Work out the finished part from the listing and answer in its coordinate system (mm). A direction names the side the tool comes from. Coordinates: 2 decimals unless noted, no trailing zeros. Order: outer loops, then holes, each group sorted by start corner. A loop starts at its lowest first (then second) coordinate and runs counter-clockwise, first axis right, second up.
```python
from build123d import *

# Parameters (mm, degrees)
SKETCH1_W           = 180
SKETCH1_H           = 50
BOSS_EXTRUDE1_DEPTH = 10
SKETCH2_W           = 10
SKETCH2_H           = 50
BOSS_EXTRUDE2_DEPTH = 16
SKETCH3_W           = 50
SKETCH3_H           = 26
CUT_EXTRUDE1_DEPTH  = 97.958754117
FILLET1_R           = 3
CHAMFER1_SIZE       = 10
SKETCH4_W           = 60
SKETCH4_H           = 50
CUT_EXTRUDE2_DEPTH  = 2


with BuildPart() as part:
    # Sketch1 → Boss-Extrude1 (new body)
    with BuildSketch(Plane(origin=(0, 0, 0), x_dir=(1, 0, 0), z_dir=(0, 1, 0))):
        Rectangle(SKETCH1_W, SKETCH1_H)
    extrude(amount=BOSS_EXTRUDE1_DEPTH)

    # Sketch2 → Boss-Extrude2 (add)
    with BuildSketch(Plane.XZ):
        with Locations((-85, 0)):
            Rectangle(SKETCH2_W, SKETCH2_H)
        with Locations((85, 0)):
            Rectangle(SKETCH2_W, SKETCH2_H)
    extrude(amount=BOSS_EXTRUDE2_DEPTH)

    # Sketch3 → Cut-Extrude1 (cut, through all)
    with BuildSketch(Plane(origin=(0, 10, 0), x_dir=(1, 0, 0), z_dir=(0, 1, 0))):
        with Locations((-65, 0)):
            Rectangle(SKETCH3_W, SKETCH3_H)
    cut_extrude1 = extrude(amount=-CUT_EXTRUDE1_DEPTH, mode=Mode.SUBTRACT)

    # Mirror1: Cut-Extrude1 across plane
    add(cut_extrude1.mirror(Plane(origin=(0, 0, 0), x_dir=(0, 0, 1), z_dir=(1, 0, 0))), mode=Mode.SUBTRACT)

    # Fillet1
    fillet1_edges = [part.edges().sort_by_distance(p)[0] for p in [
        (-40, 5, -13),
        (-40, 5, 13),
        (40, 5, 13),
        (40, 5, -13),
    ]]
    fillet(fillet1_edges, radius=FILLET1_R)

    # Chamfer1
    chamfer1_edges = [part.edges().sort_by_distance(p)[0] for p in [
        (-90, 10, -19),
        (90, 10, 19),
        (-90, 10, 19),
        (90, 10, -19),
    ]]
    chamfer(chamfer1_edges, length=CHAMFER1_SIZE)

    # Sketch4 → Cut-Extrude2 (cut)
    with BuildSketch(Plane(origin=(0, 10, 0), x_dir=(1, 0, 0), z_dir=(0, 1, 0))):
        Rectangle(SKETCH4_W, SKETCH4_H)
    extrude(amount=-CUT_EXTRUDE2_DEPTH, mode=Mode.SUBTRACT)


solid = part.part
```
1. The part is cut by section D-D (y = 5). Determine the outline of the cut face in (x, z).
2. The mould has two halves that part along X. Classify faces 5 (the flat face through (-85, -16, -19)), 6 (the cylindrical face through (40.86, 4.93, 12.1)), 7 (the flat face through (-1, 0, 0)): released by +X, released by -X, zero draft, split by the parting line, or undercut.
3. Flat-ended cylindrical pins translate along their axes: pin 1 (1.6 mm diameter, centred on y = 8.5, z = 3, fed in from -X); pin 2 (6 mm diameter, centred on x = -12.5, z = -2, fed in from -Y); pin 3 (8 mm diameter, centred on y = 5, z = -4.5, fed in from +X). Find the tip coordinate at first contact, or state that the pin passes through.
4. The part is cut by section C-C (z = 18.5). Determine the outline of the cut face in (x, y), plus the area to 3 significant figures.
5. The part is cut by section B-B (x = -73). Determine the outline of the cut face in (y, z), plus the area to 3 significant figures.
6. Consider probe 1 along Z at (x, y) = (75, 5.25); probe 2 along X at (y, z) = (-9, 22.5); probe 3 along X at (y, z) = (0.25, 5). Determine where each line is inside the solid, lowest interval first.
7. For faces 1 (the flat face through (85, -16, 19)), 2 (the cylindrical face through (-40.9, 4.93, 12.14)), 3 (the flat face through (40, 5, 0)), 4 (the flat face through (-80, -8, -19)), determine the directions among +Z, -Z, +X, -X, +Y, -Y from which every point of the face is accessible in a straight line to the end or side of a thin tool.
8. The part is cut by section A-A (y = -7.75). Determine the outline of the cut face in (x, z), plus the area to 3 significant figures.
Worked out:
1. outline: (-85, -25) - (85, -25) - (85, -13) - (43, -13) arc R3 cw to (40, -10) - (40, 10) arc R3 cw to (43, 13) - (85, 13) - (85, 25) - (-85, 25) - (-85, 13) - (-43, 13) arc R3 cw to (-40, 10) - (-40, -10) arc R3 cw to (-43, -13) - (-85, -13) - close
2. face 5: zero draft
2. face 6: released by +X
2. face 7: undercut
3. pin 1: stops at x = -40
3. pin 2: stops at y = 0
3. pin 3: stops at x = 40
4. outline: (-90, -16) - (-80, -16) - (-80, 0) - (80, 0) - (80, -16) - (90, -16) - (90, 0) - (80, 10) - (30, 10) - (30, 8) - (-30, 8) - (-30, 10) - (-80, 10) - (-90, 0) - close
4. area: 1,900 mm2
5. outline: (0, -25) - (10, -25) - (10, -13) - (0, -13) - close; (0, 13) - (10, 13) - (10, 25) - (0, 25) - close
5. area: 240 mm2
6. probe 1: z = -25 to -13, 13 to 25
6. probe 2: x = -90 to -80, 80 to 90
6. probe 3: x = -40 to 40
7. face 1: +Z, -Z, +X, -X, -Y
7. face 2: -X, +Y, -Y
7. face 3: +X, +Y, -Y
7. face 4: +Z, -Z, -Y
8. outline: (-90, -25) - (-80, -25) - (-80, -13) - (-90, -13) - close; (-90, 13) - (-80, 13) - (-80, 25) - (-90, 25) - close; (80, -25) - (90, -25) - (90, -13) - (80, -13) - close; (80, 13) - (90, 13) - (90, 25) - (80, 25) - close
8. area: 480 mm2
